Read the model definition and answer for the solid it produces. Units are mm, in the model's axes. Coordinates: 2 decimals unless noted, no trailing zeros. Order: outer loops, then holes, each group sorted by start corner. A loop starts at its lowest first (then second) coordinate and runs counter-clockwise, first axis right, second up.
from build123d import *

# Parameters (mm, degrees)
BOSS_EXTRUDE1_DEPTH = 8
FILLET1_R           = 10


with BuildPart() as part:
    # Sketch1 → Boss-Extrude1 (new body)
    with BuildSketch(Plane.XY):
        with BuildLine():
            Line((80, 125), (-80, 125))
            Line((-80, 125), (-80, 61.652250567))
            ThreePointArc((-80, 61.652250567), (0, 101), (80, 61.652250567))
            Line((80, 61.652250567), (80, 125))
        make_face()
    extrude(amount=BOSS_EXTRUDE1_DEPTH)

    # Fillet1
    fillet1_edges = [part.edges().sort_by_distance(p)[0] for p in [
        (-80, 125, 4),
        (80, 125, 4),
    ]]
    fillet(fillet1_edges, radius=FILLET1_R)


solid = part.part
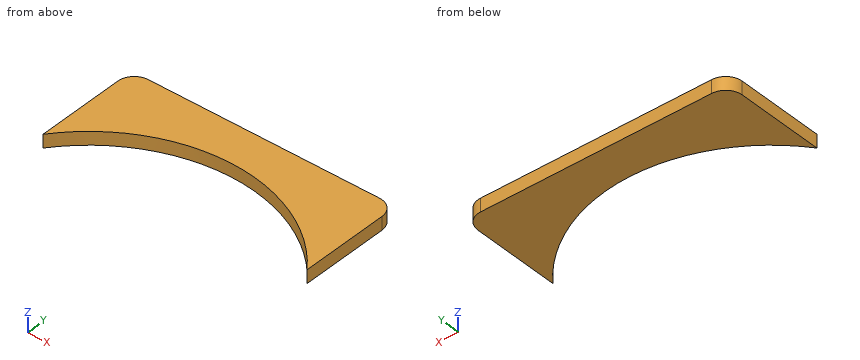
Q1. The part is cut by section C-C, the plane y = 98. Determine the outline of the cut face in (x, z), then the cut area to 3 significant figures.
Q2. Straight lines are drawn through the part: L1, parallel to X at y = 78, z = 6; L2, parallel to X at y = 74.5, z = 3.5; L3, parallel to Y at x = 51, z = 4.75. For each, find the intervals that lie inside material, in ascending order.
Q3. The part is cut by section B-B, the plane z = 2.5. Determine the outline of the cut face in (x, y), then the cut area to 3 significant figures.
Q4. The part is cut by section D-D, the plane x = -5. Determine the outline of the cut face in (y, z).
Q5. The part is cut by section A-A, the plane y = 78.5. Determine the outline of the cut face in (x, z), then the cut area to 3 significant figures.
Computed values:
1. outline: (-80, 0) - (-24.43, 0) - (-24.43, 8) - (-80, 8) - close; (24.43, 0) - (80, 0) - (80, 8) - (24.43, 8) - close
1. area: 889 mm2
2. L1: x = -80 to -64.16, 64.16 to 80
2. L2: x = -80 to -68.2, 68.2 to 80
2. L3: y = 87.18 to 125
3. outline: (-80, 61.65) arc R101 cw to (80, 61.65) - (80, 115) arc R10 ccw to (70, 125) - (-70, 125) arc R10 ccw to (-80, 115) - close
3. area: 5,700 mm2
4. outline: (100.88, 0) - (125, 0) - (125, 8) - (100.88, 8) - close
5. outline: (-80, 0) - (-63.55, 0) - (-63.55, 8) - (-80, 8) - close; (63.55, 0) - (80, 0) - (80, 8) - (63.55, 8) - close
5. area: 263 mm2
